from build123d import *

# Parameters (mm, degrees)
BASE_BLOCK_PROFILE_63X32_W  = 63
BASE_BLOCK_PROFILE_63X32_H  = 32
BASE_BLOCK_63X32X26_DEPTH   = 26
BORE_SLOT_CUT_DEPTH         = 32
RECTANGULAR_SLOT_17X9_DEPTH = 32
SIDE_STEP_PROFILE_W         = 29
SIDE_STEP_PROFILE_H         = 5
SIDE_STEP_CUT_DEPTH         = 44.866274061
SIDE_GROOVE_CUT_DEPTH       = 44.866274061


with BuildPart() as part:
    # Base Block Profile 63x32 → Base Block 63x32x26 (new body)
    with BuildSketch(Plane.XY):
        Rectangle(BASE_BLOCK_PROFILE_63X32_W, BASE_BLOCK_PROFILE_63X32_H)
    extrude(amount=BASE_BLOCK_63X32X26_DEPTH)

    # Bore Slot Profile → Bore Slot Cut (cut)
    with BuildSketch(Plane.XZ.offset(16)):
        with BuildLine():
            ThreePointArc((4.5, 26), (15.5, 15), (26.5, 26))
            Line((26.5, 26), (4.5, 26))
        make_face()
    extrude(amount=-BORE_SLOT_CUT_DEPTH, mode=Mode.SUBTRACT)

    # Rectangular Slot Profile 17x9 → Rectangular Slot 17x9 (cut)
    with BuildSketch(Plane(origin=(0, -16, 0), x_dir=(-1, 0, 0), z_dir=(0, -1, 0))):
        Polygon((31.5, -9), (14.5, -26), (31.5, -26), align=None)
    extrude(amount=-RECTANGULAR_SLOT_17X9_DEPTH, mode=Mode.SUBTRACT)

    # Side Step Profile → Side Step Cut (cut, through all)
    with BuildSketch(Plane(origin=(0, 0, 0), x_dir=(-1, 0, 0), z_dir=(0, 0, -1))):
        with Locations((17, 13.5)):
            Rectangle(SIDE_STEP_PROFILE_W, SIDE_STEP_PROFILE_H)
        with Locations((17, -13.5)):
            Rectangle(SIDE_STEP_PROFILE_W, SIDE_STEP_PROFILE_H)
    extrude(amount=-SIDE_STEP_CUT_DEPTH, mode=Mode.SUBTRACT)

    # Side Groove Profile → Side Groove Cut (cut, through all)
    with BuildSketch(Plane(origin=(0, 0, 0), x_dir=(-1, 0, 0), z_dir=(0, 0, -1))):
        Polygon((31.5, -5.002946395), (31.5, 0), (31.5, 5), (2.592435859, 5), (2.592435859, -5.002946395), align=None)
    extrude(amount=-SIDE_GROOVE_CUT_DEPTH, mode=Mode.SUBTRACT)


solid = part.part
Design review of the part built by this model. Coordinates are the model's own, in mm. A direction names the side the tool comes from. Coordinates: 2 decimals unless noted, no trailing zeros. Order: outer loops, then holes, each group sorted by start corner. A loop starts at its lowest first (then second) coordinate and runs counter-clockwise, first axis right, second up. Notation, with made-up numbers: (71, 48) - (99, 48) arc R31 cw to (99, 78) - close; hole circle Ø11 at (-32, 73.5). An arc over 180 degrees is marked (long way). Put each result on its own line as item: value.
1) Take a section at C-C, the plane y = -8. Give the boundary of the cut face in (x, z).
Response values:
outline: (-31.5, 0) - (31.5, 0) - (31.5, 26) - (26.5, 26) arc R11 cw to (4.5, 26) - (-14.5, 26) - (-31.5, 9) - close
2) Take a section at A-A, the plane x = -6.5. Give the boundary of the cut face in (y, z), and give its area (3 significant figures).
Response values:
outline: (-11, 0) - (-5, 0) - (-5, 26) - (-11, 26) - close; (5, 0) - (11, 0) - (11, 26) - (5, 26) - close
area: 312 mm²
3) Insertion check: P1, Ø8, axis at x = -19.5, z = 15.5, coming from the -Y side; P2, Ø2.5, axis at y = -12.5, z = 9.5, coming from the -X side; P3, Ø5, axis at y = 0.5, z = 10, coming from the -X side. Each pin has a flat end and moves straight along its axis. Give the tip position at first contact, or say it passes through.
Response values:
P1: stops at y = -11
P2: stops at x = -2.5
P3: stops at x = -2.59
4) Take a section at D-D, the plane z = 4. Give the boundary of the cut face in (x, y), and give its area (3 significant figures).
Response values:
outline: (-31.5, -11) - (-2.5, -11) - (-2.5, -16) - (31.5, -16) - (31.5, 16) - (-2.5, 16) - (-2.5, 11) - (-31.5, 11) - (-31.5, 5) - (-2.59, 5) - (-2.59, -5) - (-31.5, -5) - close
area: 1,440 mm²
5) The part is to be moulded in two halves that separate along Y. For faces 1 (the face through (-14, -5.003, 10)), 2 (the face through (31.5, 0, 13)), 3 (the face through (-14, -11, 10)), say which applies: released by +Y, released by -Y, zero draft, split by the parting line, or undercut.
Response values:
face 1: undercut
face 2: zero draft
face 3: released by -Y
6) Wall thickness on L1, parallel to Y at x = -25, z = 10; L2, parallel to X at y = 11.5, z = 1; L3, parallel to Z at x = -24.5, y = 9: over which ranges is each line inside the solid? List them lowest first. Write a range as from..to.
Response values:
L1: y = -11..-5, 5..11
L2: x = -2.5..31.5
L3: z = 0..16
7) Take a section at B-B, the plane z = 17. Give the boundary of the cut face in (x, y), and give its area (3 significant figures).
Response values:
outline: (-23.5, -11) - (-2.5, -11) - (-2.5, -16) - (9.18, -16) - (9.18, 16) - (-2.5, 16) - (-2.5, 11) - (-23.5, 11) - (-23.5, 5) - (-2.59, 5) - (-2.59, -5) - (-23.5, -5) - close; (21.82, -16) - (31.5, -16) - (31.5, 16) - (21.82, 16) - close
area: 936 mm²
8) Tool access review of faces 4 (the face through (7, 0, 0)), 5 (the face through (-31.5, -8, 4)), 6 (the face through (-2.5, -14, 13)), 7 (the face through (-2.592, 0, 13)), 8 (the face through (-2.5, 13, 13)): name each direction out of +Z, -Z, +X, -X, +Y, -Y from which nothing blocks a thin tool from reaching the whole face with its end or side.
Response values:
face 4: -Z, +X, -X, +Y, -Y
face 5: +Z, -Z, -X, +Y, -Y
face 6: +Z, -Z, -X, -Y
face 7: +Z, -Z, -X
face 8: +Z, -Z, -X, +Y
